For this review, take the finished solid that the model builds, in its own axes (mm). Coordinates: 2 decimals unless noted, no trailing zeros. Loops run counter-clockwise (first coordinate to the right, second up) from the corner with the lowest first, then second, coordinate; pieces in that order, holes last. Notation, with made-up numbers: M 75,15 L 125,15 A22 ccw 125,51 Z; hole C 30,67 d3. An arc over 180 degrees is marked long. Answer as a JSON object with one key per item and string values. Group by question number.
Item 1: Insertion check: pin 1 (1 mm diameter, centred on y = -61.5, z = 2, fed in from -X); pin 2 (2 mm diameter, centred on y = -28.5, z = 2.5, fed in from -X). Each pin has a flat end and moves straight along its axis. Give the tip position at first contact, or say it passes through.
Item 2: Add section B-B (x = -6.5). State the section outline as (y, z) points, then the cut area to 3 significant figures.
Item 3: Wall thickness on L1, parallel to X at y = -155.5, z = 2.1; L2, parallel to X at y = -77.5, z = 3.5: over which ranges is each line inside the solid? List them lowest first. Write a range as from..to.
Item 4: Add section A-A (z = 0.8). State the section outline as (x, y) points, then the cut area to 3 significant figures.
Item 5: Add section C-C (y = -17). State the section outline as (x, z) points, then the cut area to 3 significant figures.
from build123d import *

# Parameters (mm, degrees)
BOSS_EXTRUDE1_DEPTH = 5


with BuildPart() as part:
    # Sketch1 → Boss-Extrude1 (new body)
    with BuildSketch(Plane.XY):
        with BuildLine():
            Line((0, 0), (-50, -184))
            Line((-50, -184), (-50, -192))
            Line((-50, -192), (37, -192))
            ThreePointArc((37, -192), (40.535533906, -190.535533906), (42, -187))
            Line((42, -187), (42, 0))
            Line((42, 0), (0, 0))
        make_face()
    extrude(amount=BOSS_EXTRUDE1_DEPTH)


solid = part.part
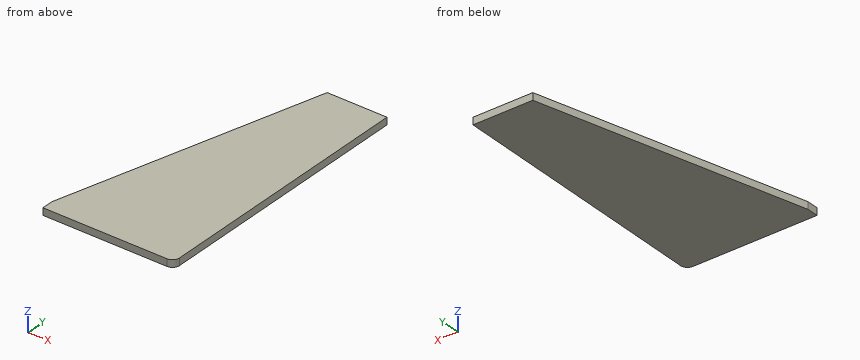
From the geometry:
{
 "1": {"pin 1": "stops at x = -16.85", "pin 2": "stops at x = -8.02"},
 "2": {"outline": "M -192,0 L -23.92,0 L -23.92,5 L -192,5 Z", "area": "840 mm²"},
 "3": {"L1": "x = -42.26..42", "L2": "x = -21.06..42"},
 "4": {"outline": "M -50,-192 L 37,-192 A5 ccw 42,-187 L 42,0 L 0,0 L -50,-184 Z", "area": "13,100 mm²"},
 "5": {"outline": "M -4.62,0 L 42,0 L 42,5 L -4.62,5 Z", "area": "233 mm²"}
}
